Geometry: final body of the model. Coordinates: model frame, mm. A direction names the side the tool comes from. Coordinates: 2 decimals unless noted, no trailing zeros. Loops run counter-clockwise (first coordinate to the right, second up) from the corner with the lowest first, then second, coordinate; pieces in that order, holes last. Notation, with made-up numbers: M 46,10 L 89,10 A21 ccw 89,16 Z; hole C 60,21.5 d7. An arc over 180 degrees is marked long. Write each question's results on one line, items separated by ' | '. Start each with the question number.
from build123d import *

# Parameters (mm, degrees)
SKETCH_1_W          = 120
SKETCH_1_H          = 50
EXTRUDE_1_DEPTH     = 60
SKETCH_2_R          = 42.5
CUT_EXTRUDE_1_DEPTH = 60
SKETCH_3_W          = 30
SKETCH_3_H          = 50
EXTRUDE_2_DEPTH     = 20
FILLET_1_R          = 10
EXTRUDE_START       = 3
EXTRUDE_3_DEPTH     = 3
SKETCH_5_R          = 6
CUT_EXTRUDE_2_DEPTH = 67


with BuildPart() as part:
    # 草图1 → 凸台-拉伸1 (new body)
    with BuildSketch(Plane(origin=(0, 0, 0), x_dir=(1, 0, 0), z_dir=(0, 1, 0))):
        Rectangle(SKETCH_1_W, SKETCH_1_H)
    extrude(amount=EXTRUDE_1_DEPTH)

    # 草图2 → 切除-拉伸1 (cut)
    with BuildSketch(Plane.XY.offset(25)):
        Circle(SKETCH_2_R)
    extrude(amount=-CUT_EXTRUDE_1_DEPTH, mode=Mode.SUBTRACT)

    # 草图3 → 凸台-拉伸2 (add)
    with BuildSketch(Plane.XZ):
        with Locations((-75, 0)):
            Rectangle(SKETCH_3_W, SKETCH_3_H)
        with Locations((75, 0)):
            Rectangle(SKETCH_3_W, SKETCH_3_H)
    extrude(amount=-EXTRUDE_2_DEPTH)

    # 圆角1
    fillet_1_edges = [part.edges().sort_by_distance(p)[0] for p in [
        (-60, 60, 0),
        (60, 60, 0),
    ]]
    fillet(fillet_1_edges, radius=FILLET_1_R)

    # 草图4 → 凸台-拉伸3 (add)
    with BuildSketch(Plane.XY.offset(25).offset(EXTRUDE_START)):
        with BuildLine():
            Line((-52.5, 0), (-42.5, 0))
            ThreePointArc((-42.5, 0), (0, 42.5), (42.5, 0))
            Line((42.5, 0), (52.5, 0))
            ThreePointArc((52.5, 0), (0, 52.5), (-52.5, 0))
        make_face()
    extrude_3 = extrude(amount=-EXTRUDE_3_DEPTH)

    # 镜向1: 凸台-拉伸3 across plane
    add(extrude_3.mirror(Plane.XY))

    # 草图5 → 切除-拉伸2 (cut)
    with BuildSketch(Plane(origin=(0, 20, 0), x_dir=(1, 0, 0), z_dir=(0, 1, 0))):
        with Locations(Location((75, 12.5, 0), (0, 0, 270))):
            Circle(SKETCH_5_R)
        with Locations(Location((75, -12.5, 0), (0, 0, 270))):
            Circle(SKETCH_5_R)
        with Locations(Location((-75, -12.5, 0), (0, 0, 270))):
            Circle(SKETCH_5_R)
        with Locations(Location((-75, 12.5, 0), (0, 0, 270))):
            Circle(SKETCH_5_R)
    extrude(amount=-CUT_EXTRUDE_2_DEPTH, mode=Mode.SUBTRACT)


solid = part.part
Item 1: Section B-B, the plane x = 0. Return loops of the section in (y, z), plus the area to 3 significant figures.
Item 2: Contact query for flat-ended pins moving along their axis: P1, Ø14, axis at x = -75, z = -12.5, coming from the +Y side; P2, Ø8, axis at y = 35.5, z = -3, coming from the -X side; P3, Ø3, axis at x = -34.5, z = 21, coming from the -Y side. Output: stop coordinate, or through.
Item 3: Set-up query: faces 1 (the flat face through (-75, 20, 0)), 2 (the cylindrical face through (-69.941, 10.14, -9.274)), 3 (the flat face through (8, 42, 28)), 4 (the cylindrical face through (1.154, 52.487, 26.521)), 5 (the cylindrical face through (1.154, 52.487, -26.521)). Return all of +Z, -Z, +X, -X, +Y, -Y with unobstructed straight access to the full face (end or side cutting, diameter ignored); none if empty.
Item 4: Section D-D, the plane z = -22. Return loops of the section in (x, y).
Item 5: Ray query, L1, parallel to X at y = 10, z = 12.5; L2, parallel to X at y = 14, z = 12; L3, parallel to X at y = 48, z = 5. Return the intervals inside material, ascending. Write a range as [from, to].
Item 6: Section C-C, the plane y = 38.5. Return loops of the section in (x, z), plus the area to 3 significant figures.
Item 7: Section A-A, the plane z = -12.5. Return loops of the section in (x, y), plus the area to 3 significant figures.
Item 8: Pull-direction query (Z, two-part tool) for faces 6 (the flat face through (8, 42, -28)), 7 (the flat face through (-60, 35, 0)), 8 (the cylindrical face through (80.059, 10.14, 15.726)); classes: released by +Z, released by -Z, zero draft, split by the parting line, or undercut.
Solutions:
1) outline: M 42.5,-28 L 52.5,-28 L 52.5,-25 L 60,-25 L 60,25 L 52.5,25 L 52.5,28 L 42.5,28 Z | area: 935 mm²
2) P1: stops at y = 20 | P2: stops at x = -60 | P3: stops at y = 22.59
3) face 1: +Z, -Z, -X, +Y | face 2: +Y, -Y | face 3: +Z, +X, -X, +Y, -Y | face 4: +Z, +Y | face 5: -Z, +Y
4) outline: M -90,0 L -42.5,0 A42.5 cw 42.5,0 L 90,0 L 90,20 L 60,20 L 60,50 A10 ccw 50,60 L -50,60 A10 ccw -60,50 L -60,20 L -90,20 Z
5) L1: x = [-90, -81], [-69, -41.31], [41.31, 69], [81, 90] | L2: x = [-90, -80.98], [-69.02, -40.13], [40.13, 69.02], [80.98, 90] | L3: x = [-60, 60]
6) outline: M -60,-25 L -35.69,-25 L -35.69,-28 L -18,-28 L -18,28 L -35.69,28 L -35.69,25 L -60,25 Z; M 18,-28 L 35.69,-28 L 35.69,-25 L 60,-25 L 60,25 L 35.69,25 L 35.69,28 L 18,28 Z | area: 4,410 mm²
7) outline: M -90,0 L -81,0 L -81,20 L -90,20 Z; M -69,0 L -42.5,0 A42.5 cw 42.5,0 L 69,0 L 69,20 L 60,20 L 60,50 A10 ccw 50,60 L -50,60 A10 ccw -60,50 L -60,20 L -69,20 Z; M 81,0 L 90,0 L 90,20 L 81,20 Z | area: 5,040 mm²
8) face 6: released by -Z | face 7: zero draft | face 8: undercut
